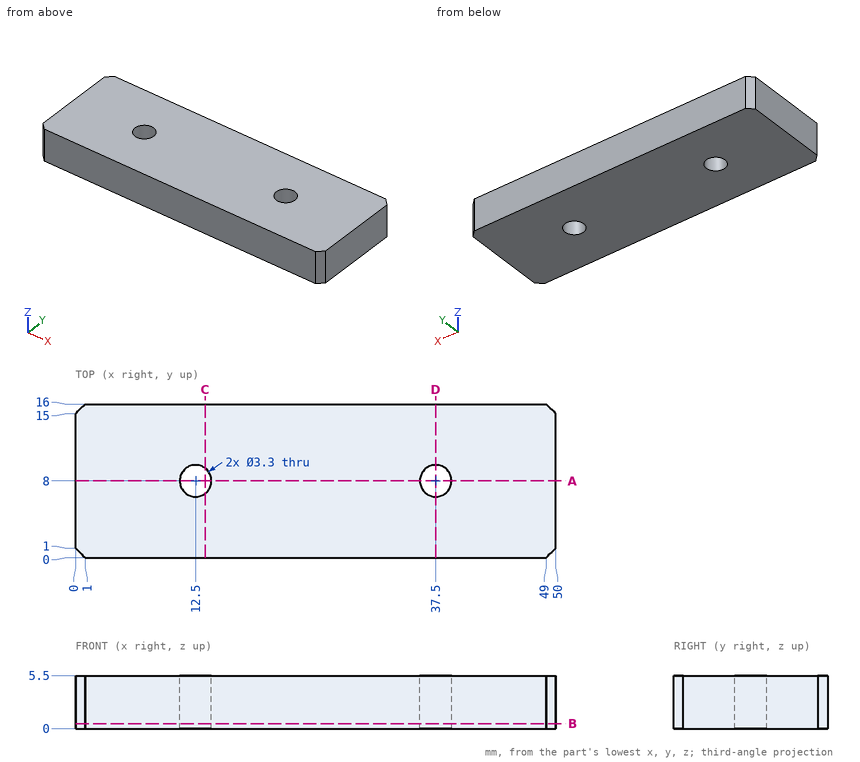
Input: dimensioned drawing with shaded views. Units: mm. Origin: part minimum x, y, z. Give positions to 0.01 mm unless a question says otherwise; leave off trailing zeros. Order: outer loops, then holes, each group sorted by start corner. A loop starts at its lowest first (then second) coordinate and runs counter-clockwise, first axis right, second up. Notation, with made-up numbers: (66, -39.75) -> (105, -39.75) arc R21 ccw to (105, -7.75) -> close; hole circle Ø11 at (-39, 15.25). An arc over 180 degrees is marked (long way). Use one line per item in the form item = value.
1) Line query: probe 1 along Y at (x, z) = (12.5, 3.75); probe 2 along X at (y, z) = (8.75, 2.3). Output: solid intervals per line, ascending.
Response values:
probe_1 = 0 to 6.35, 9.65 to 16
probe_2 = 0 to 11.03, 13.97 to 36.03, 38.97 to 50
2) Section A-A, the plane y = 8. Return loops of the section in (x, z), and give its area (3 significant figures).
Response values:
outline = (0, 0) -> (10.85, 0) -> (10.85, 5.5) -> (0, 5.5) -> close; (14.15, 0) -> (35.85, 0) -> (35.85, 5.5) -> (14.15, 5.5) -> close; (39.15, 0) -> (50, 0) -> (50, 5.5) -> (39.15, 5.5) -> close
area = 239 mm^2
3) Section C-C, the plane x = 13.5. Return loops of the section in (y, z), and give its area (3 significant figures).
Response values:
outline = (0, 0) -> (6.69, 0) -> (6.69, 5.5) -> (0, 5.5) -> close; (9.31, 0) -> (16, 0) -> (16, 5.5) -> (9.31, 5.5) -> close
area = 73.6 mm^2
4) Section D-D, the plane x = 37.5. Return loops of the section in (y, z).
Response values:
outline = (0, 0) -> (6.35, 0) -> (6.35, 5.5) -> (0, 5.5) -> close; (9.65, 0) -> (16, 0) -> (16, 5.5) -> (9.65, 5.5) -> close
5) Section B-B, the plane z = 0.5. Return loops of the section in (x, y), and give its area (3 significant figures).
Response values:
outline = (0, 1) -> (1, 0) -> (49, 0) -> (50, 1) -> (50, 15) -> (49, 16) -> (1, 16) -> (0, 15) -> close; hole circle Ø3.3 at (12.5, 8); hole circle Ø3.3 at (37.5, 8)
area = 781 mm^2
